```python
from build123d import *

# Parameters (mm, degrees)
SKETCH1_W                   = 80
SKETCH1_H                   = 80
BOSS_EXTRUDE1_DEPTH         = 24
HOLE1_D                     = 33
HOLE1_CBORE_D               = 49
HOLE1_CBORE_DEPTH           = 12
M8_TAPPED_HOLE1_D           = 6.8
M8_TAPPED_HOLE1_CSINK_D     = 8.05
M8_TAPPED_HOLE1_CSINK_ANGLE = 90
CHAMFER1_SIZE               = 5


with BuildPart() as part:
    # Sketch1 → Boss-Extrude1 (new body)
    with BuildSketch(Plane.XY):
        with Locations((-12.568836811, 18.618181818)):
            Rectangle(SKETCH1_W, SKETCH1_H)
    extrude(amount=BOSS_EXTRUDE1_DEPTH)

    # Hole1 (through all)
    with Locations(Plane.XY.offset(24)):
        with Locations((-12.568836811, 18.618181818)):
            CounterBoreHole(HOLE1_D / 2, HOLE1_CBORE_D / 2, HOLE1_CBORE_DEPTH)

    # M8 Tapped Hole1 (through all)
    with Locations(Plane.XY.offset(24)):
        with Locations((-41.568836811, 47.618181818), (16.431163189, 47.618181818), (16.431163189, -10.381818182), (-41.568836811, -10.381818182)):
            CounterSinkHole(M8_TAPPED_HOLE1_D / 2, M8_TAPPED_HOLE1_CSINK_D / 2, counter_sink_angle=M8_TAPPED_HOLE1_CSINK_ANGLE)

    # Chamfer1
    chamfer1_edges = [part.edges().sort_by_distance(p)[0] for p in [
        (-52.568836811, 58.618181818, 12),
        (27.431163189, 58.618181818, 12),
        (27.431163189, -21.381818182, 12),
        (-52.568836811, -21.381818182, 12),
    ]]
    chamfer(chamfer1_edges, length=CHAMFER1_SIZE)


solid = part.part
```
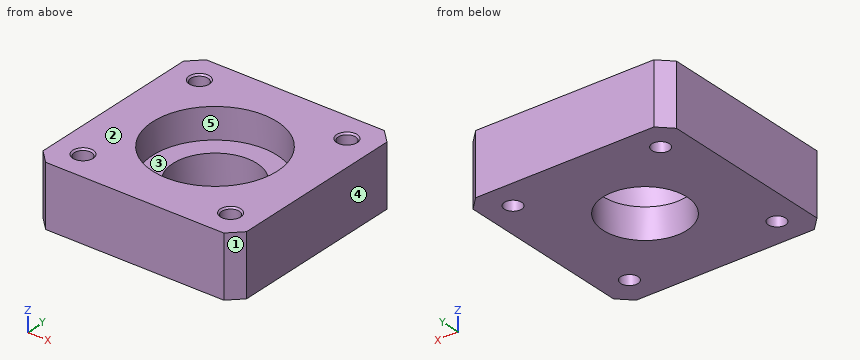
For this review, take the finished solid that the model builds, in its own axes (mm). Face numbers are marked on the shaded views. A direction names the side the tool comes from. Round coordinates to 2 decimals unless told otherwise and drop trailing zeros. Write each loop counter-clockwise with the first axis right and the second up, starting at its lowest first coordinate (ties: lowest second). Pieces come first, ordered by that corner, then holes.
1) Machinability: for the marked faces 4 and 5, which of the approach directions +Z, -Z, +X, -X, +Y, -Y give a long, thin tool a straight path to every point of the face, cutting with its end or side? Answer none if there is none.
Answer below:
face 4: +Z, -Z, +X, +Y, -Y
face 5: +Z
2) Take a section at A-A on x = -11. Give the boundary of the cut face in (y, z).
Answer below:
outline: (-21.38, 0) - (2.19, 0) - (2.19, 12) - (-5.83, 12) - (-5.83, 24) - (-21.38, 24) - close; (35.04, 0) - (58.62, 0) - (58.62, 24) - (43.07, 24) - (43.07, 12) - (35.04, 12) - close
3) Take a section at B-B on y = 9.5. Give the boundary of the cut face in (x, z).
Answer below:
outline: (-52.57, 0) - (-26.32, 0) - (-26.32, 12) - (-35.31, 12) - (-35.31, 24) - (-52.57, 24) - close; (1.18, 0) - (27.43, 0) - (27.43, 24) - (10.17, 24) - (10.17, 12) - (1.18, 12) - close
4) Mouldability with a two-part tool opening along Y and no side actions: class the marked faces 1, 2 and 3 as +Y half, -Y half, draft (parallel to the pull), parting line (faces both ways), or undercut.
Answer below:
face 1: -Y half
face 2: draft
face 3: undercut
5) Insertion check: pin 1 Ø5.5 at (x, y) = (16.43, 47.62) entering from +Z; pin 2 Ø4 at (x, y) = (-11.5, 36.5) entering from +Z. Each pin has a flat end and moves straight along its axis. Give the tip position at first contact, or say it passes through.
Answer below:
pin 1: passes through
pin 2: stops at z = 12
6) For line 1 along Y through (x, z) = (19, 17.25); line 2 along X through (y, z) = (-13, 6.5); line 3 along Y through (x, z) = (15, 19.5), list the stretches that pass through material, from the lowest coordinate up.
Answer below:
line 1: y = -21.38 to -12.61, -8.15 to 45.39, 49.85 to 58.62
line 2: x = -52.57 to -43.74, -39.4 to 14.26, 18.6 to 27.43
line 3: y = -21.38 to -13.47, -7.3 to 44.53, 50.7 to 58.62
7) Take a section at D-D on x = -34.5. Give the boundary of the cut face in (y, z), then the cut area to 3 significant figures.
Answer below:
outline: (-21.38, 0) - (58.62, 0) - (58.62, 24) - (29.54, 24) - (29.54, 12) - (7.7, 12) - (7.7, 24) - (-21.38, 24) - close
area: 1,660 mm2
8) Take a section at C-C on z = 17.25. Give the boundary of the cut face in (x, y), then the cut area to 3 significant figures.
Answer below:
outline: (-52.57, -16.38) - (-47.57, -21.38) - (22.43, -21.38) - (27.43, -16.38) - (27.43, 53.62) - (22.43, 58.62) - (-47.57, 58.62) - (-52.57, 53.62) - close; hole circle Ø6.8 at (-41.57, -10.38); hole circle Ø6.8 at (-41.57, 47.62); hole circle Ø49 at (-12.57, 18.62); hole circle Ø6.8 at (16.43, -10.38); hole circle Ø6.8 at (16.43, 47.62)
area: 4,320 mm2
